Here's the drawing with two shaded views (mm, measured from the low corner). I have some questions. A direction names the side the tool comes from. Give positions to 0.01 mm unless a question says otherwise; leave off trailing zeros. Write each loop counter-clockwise with the first axis right and the second up, starting at its lowest first coordinate (ties: lowest second). Pieces come first, ordered by that corner, then holes. Notation, with made-up numbers: (37.5, 33.5) - (82.5, 33.5) arc R19 cw to (82.5, 43.5) - close; hole circle Ø3 at (83.25, 3). An arc over 180 degrees is marked (long way). Use one line per item in the form item = value.
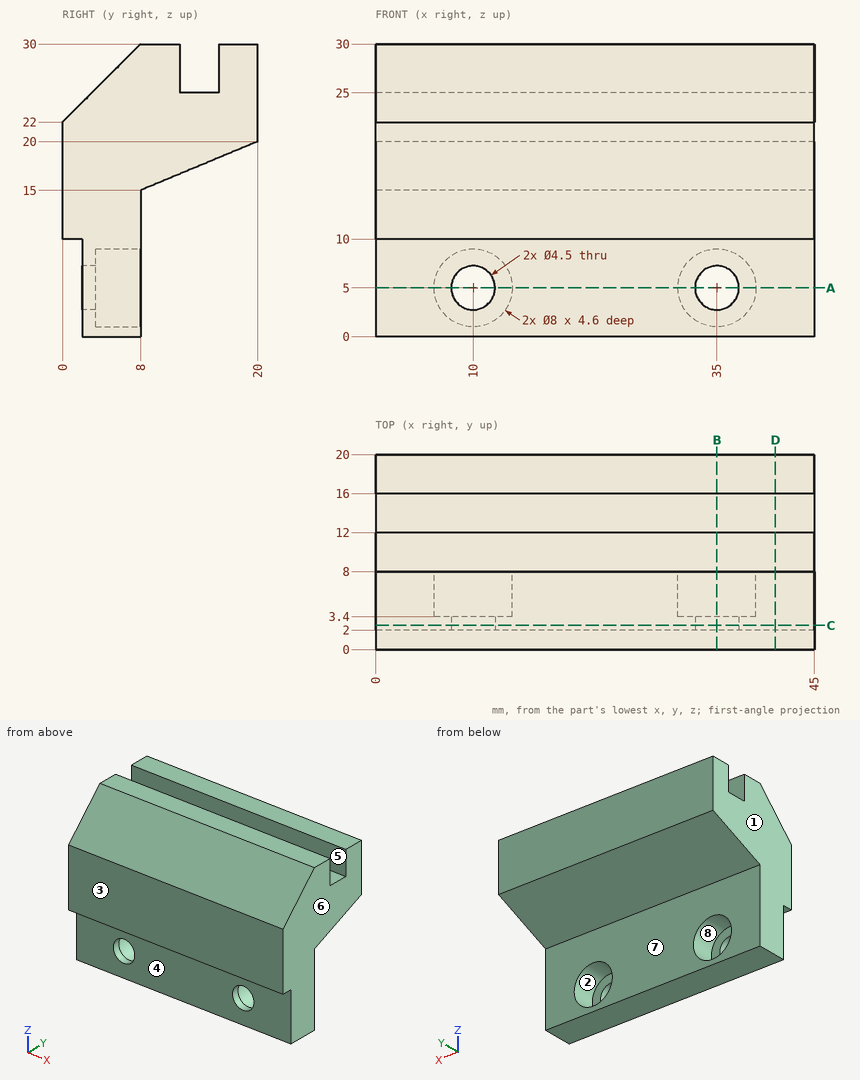
1. If I drill on line 1 (Z direction, x = 9, y = 7.5); line 2 (Y direction, x = 22.5, z = 5.75); line 3 (Y direction, x = 6, z = 11.5), over which ranges is the centre line in solid material (lowest first)? Write a range as from..to.
Response values:
line_1 = 0..1.13, 8.87..29.5
line_2 = 2..8
line_3 = 0..8
2. Imagine slicing it at C-C, the plane y = 2.5. List the corners of the cut face in (x, z) for me, and give its area (3 significant figures).
Response values:
outline = (0, 0) - (45, 0) - (45, 24.5) - (0, 24.5) - close; hole circle Ø4.5 at (10, 5); hole circle Ø4.5 at (35, 5)
area = 1,070 mm²
3. For pin 1 (6.5 mm diameter, centred on x = 36, z = 6.5, fed in from +Y); pin 2 (5 mm diameter, centred on x = 16.5, z = 6, fed in from -Y); pin 3 (1.5 mm diameter, centred on x = 13, z = 27, fed in from -Y), each with a flat end and sliding along its axis, tell me the tip position at first contact or that it passes through.
Response values:
pin_1 = 8
pin_2 = 2
pin_3 = 4.25
4. Which directions (+Z, -Z, +X, -X, +Y, -Y) give clear straight access to the entire face, cutting with the end or side of a thin tool? Please do the marked faces 4, 5, 6, 7 and 8.
Response values:
face_4 = -Z, +X, -X, -Y
face_5 = +Z, +X, -X
face_6 = +Z, -Z, +X, +Y, -Y
face_7 = -Z, +X, -X, +Y
face_8 = +Y
5. Imagine slicing it at D-D, the plane x = 41. List the corners of the cut face in (y, z) for me.
Response values:
outline = (0, 10) - (2, 10) - (2, 0) - (8, 0) - (8, 15) - (20, 20) - (20, 30) - (16, 30) - (16, 25) - (12, 25) - (12, 30) - (8, 30) - (0, 22) - close
6. Imagine slicing it at A-A, the plane z = 5. List the corners of the cut face in (x, y) for me, and give its area (3 significant figures).
Response values:
outline = (0, 2) - (7.75, 2) - (7.75, 3.4) - (6, 3.4) - (6, 8) - (0, 8) - close; (12.25, 2) - (32.75, 2) - (32.75, 3.4) - (31, 3.4) - (31, 8) - (14, 8) - (14, 3.4) - (12.25, 3.4) - close; (37.25, 2) - (45, 2) - (45, 8) - (39, 8) - (39, 3.4) - (37.25, 3.4) - close
area = 184 mm²
7. If we mould it in two halves opening along X, with no side actions, what happens to the marked faces 1, 2 and 3? For each: pulls with the +X half, pulls with the -X half, needs draft (parallel to the pull), parting line crosses it, or undercut.
Response values:
face_1 = pulls with the -X half
face_2 = undercut
face_3 = needs draft
8. Imagine slicing it at B-B, the plane x = 35. List the corners of the cut face in (y, z) for me, and give its area (3 significant figures).
Response values:
outline = (0, 10) - (2, 10) - (2, 7.25) - (3.4, 7.25) - (3.4, 9) - (8, 9) - (8, 15) - (20, 20) - (20, 30) - (16, 30) - (16, 25) - (12, 25) - (12, 30) - (8, 30) - (0, 22) - close; (2, 0) - (8, 0) - (8, 1) - (3.4, 1) - (3.4, 2.75) - (2, 2.75) - close
area = 275 mm²
